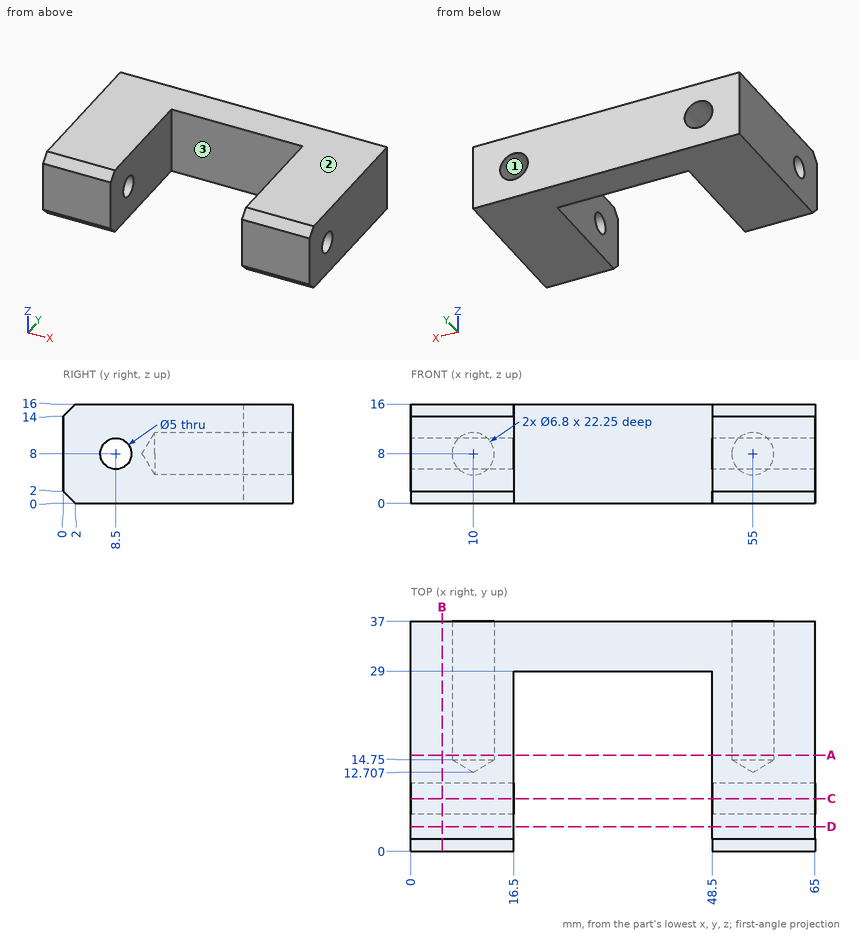
Answer from the drawing. Dimensions are ordinates in mm from the lowest x, y and z of the part. A direction names the side the tool comes from. Coordinates: 2 decimals unless noted, no trailing zeros. Loops run counter-clockwise (first coordinate to the right, second up) from the corner with the lowest first, then second, coordinate; pieces in that order, holes last. Notation, with made-up numbers: (82, 73) - (139, 73) arc R16 ccw to (139, 98) - close; hole circle Ø6 at (15.5, -24). An arc over 180 degrees is marked (long way). Answer in a Markdown table with one row per item.
1. Find section D-D, the plane y = 4. Write down the section's boundary in (x, z), then the cut area to 3 significant figures.
Conclusion:
| item | result |
|---|---|
| outline | (0, 0) - (16.5, 0) - (16.5, 16) - (0, 16) - close; (48.5, 0) - (65, 0) - (65, 16) - (48.5, 16) - close |
| area | 528 mm² |
2. Straight lines are drawn through the part: line 1 (X direction, y = 31, z = 8); line 2 (Y direction, x = 58.5, z = 8); line 3 (X direction, y = 24, z = 2.5). For each, find the intervals that lie inside material, in ascending order.
Conclusion:
| item | result |
|---|---|
| line 1 | x = 0 to 6.6, 13.4 to 51.6, 58.4 to 65 |
| line 2 | y = 0 to 6, 11 to 37 |
| line 3 | x = 0 to 16.5, 48.5 to 65 |
3. Given pin 1 (3 mm diameter, centred on y = 8.5, z = 8, fed in from -X), flat-ended and moving along its own axis, determine where the tip first touches the part or whether it passes through.
Conclusion:
| item | result |
|---|---|
| pin 1 | passes through |
4. Find section A-A, the plane y = 15.5. Write down the section's boundary in (x, z), then the cut area to 3 significant figures.
Conclusion:
| item | result |
|---|---|
| outline | (0, 0) - (16.5, 0) - (16.5, 16) - (0, 16) - close; (48.5, 0) - (65, 0) - (65, 16) - (48.5, 16) - close; hole circle Ø6.8 at (10, 8); hole circle Ø6.8 at (55, 8) |
| area | 455 mm² |
5. Find section B-B, the plane x = 5. Write down the section's boundary in (y, z).
Conclusion:
| item | result |
|---|---|
| outline | (0, 2) - (2, 0) - (37, 0) - (37, 16) - (2, 16) - (0, 14) - close; hole circle Ø5 at (8.5, 8) |
6. Which of the six approach directions +Z, -Z, +X, -X, +Y, -Y give full straight-line access (tool end or side, diameter ignored) to the marked faces 1, 2 and 3?
Conclusion:
| item | result |
|---|---|
| face 1 | +Y |
| face 2 | +Z, +X, -X, +Y, -Y |
| face 3 | +Z, -Z, -Y |
7. Find section C-C, the plane y = 8.5. Write down the section's boundary in (x, z), then the cut area to 3 significant figures.
Conclusion:
| item | result |
|---|---|
| outline | (0, 0) - (16.5, 0) - (16.5, 5.5) - (0, 5.5) - close; (0, 10.5) - (16.5, 10.5) - (16.5, 16) - (0, 16) - close; (48.5, 0) - (65, 0) - (65, 5.5) - (48.5, 5.5) - close; (48.5, 10.5) - (65, 10.5) - (65, 16) - (48.5, 16) - close |
| area | 363 mm² |
